```python
from build123d import *

# Parameters (mm, degrees)
BOSS_EXTRUDE1_DEPTH     = 240
CUT_EXTRUDE1_DEPTH      = 263.392835268
CUT_EXTRUDE2_DEPTH      = 263.392835268
CUT_EXTRUDE2_DEPTH_BACK = 263.392835268
SKETCH2_R               = 17.5
CHAMFER1_SIZE           = 4


with BuildPart() as part:
    # Sketch1 → Boss-Extrude1 (new, symmetric)
    with BuildSketch(Plane.XY):
        with BuildLine():
            Line((-63, -75), (63, -75))
            ThreePointArc((63, -75), (71.485281374, -71.485281374), (75, -63))
            Line((75, -63), (75, 63))
            ThreePointArc((75, 63), (71.485281374, 71.485281374), (63, 75))
            Line((63, 75), (-63, 75))
            ThreePointArc((-63, 75), (-71.485281374, 71.485281374), (-75, 63))
            Line((-75, 63), (-75, -63))
            ThreePointArc((-75, -63), (-71.485281374, -71.485281374), (-63, -75))
        make_face()
        with BuildLine():
            Line((-63, -69), (63, -69))
            ThreePointArc((63, -69), (67.242640687, -67.242640687), (69, -63))
            Line((69, -63), (69, 63))
            ThreePointArc((69, 63), (67.242640687, 67.242640687), (63, 69))
            Line((63, 69), (-63, 69))
            ThreePointArc((-63, 69), (-67.242640687, 67.242640687), (-69, 63))
            Line((-69, 63), (-69, -63))
            ThreePointArc((-69, -63), (-67.242640687, -67.242640687), (-63, -69))
        make_face(mode=Mode.SUBTRACT)
    extrude(amount=BOSS_EXTRUDE1_DEPTH, both=True)

    # 草图1 → Cut-Extrude1 (cut, through all)
    with BuildSketch(Plane(origin=(0, 0, 0), x_dir=(1, 0, 0), z_dir=(0, 1, 0))):
        with BuildLine():
            Line((40, -290), (-40, -290))
            Line((-40, -290), (-40, -200))
            ThreePointArc((-40, -200), (-37.071067812, -192.928932188), (-30, -190))
            Line((-30, -190), (30, -190))
            ThreePointArc((30, -190), (37.071067812, -192.928932188), (40, -200))
            Line((40, -200), (40, -290))
        make_face()
    extrude(amount=CUT_EXTRUDE1_DEPTH, mode=Mode.SUBTRACT)

    # Sketch2 → Cut-Extrude2 (cut, two sides: drawn at the far end of the back side and taken through both)
    with BuildSketch(Plane(origin=(0, 0, 0), x_dir=(0, 0, -1), z_dir=(1, 0, 0)).offset(-CUT_EXTRUDE2_DEPTH_BACK)):
        with Locations((-210, 0)):
            Circle(SKETCH2_R)
        with BuildLine():
            Line((200, 35), (285, 35))
            Line((285, 35), (285, -35))
            Line((285, -35), (200, -35))
            ThreePointArc((200, -35), (196.464466094, -33.535533906), (195, -30))
            Line((195, -30), (195, 30))
            ThreePointArc((195, 30), (196.464466094, 33.535533906), (200, 35))
        make_face()
    extrude(amount=CUT_EXTRUDE2_DEPTH + CUT_EXTRUDE2_DEPTH_BACK, mode=Mode.SUBTRACT)

    # Chamfer1
    chamfer1_edges = [part.edges().sort_by_distance(p)[0] for p in [
        (-67.242640687, 67.242640687, -240),
        (-69, 49, -240),
        (-67.242640687, -67.242640687, -240),
        (0, -69, -240),
        (67.242640687, -67.242640687, -240),
        (69, -49, -240),
        (67.242640687, 67.242640687, -240),
        (0, 69, -240),
        (69, 49, -240),
        (-69, -49, -240),
    ]]
    chamfer(chamfer1_edges, length=CHAMFER1_SIZE)


solid = part.part
```
Design review of the part built by this model. Coordinates are the model's own, in mm. A direction names the side the tool comes from. Round coordinates to 2 decimals unless told otherwise and drop trailing zeros. Order: outer loops, then holes, each group sorted by start corner. A loop starts at its lowest first (then second) coordinate and runs counter-clockwise, first axis right, second up. Notation, with made-up numbers: (13.25, 30.25) - (72.25, 30.25) arc R19 cw to (72.25, 55.25) - close; hole circle Ø5 at (-15, 88). An arc over 180 degrees is marked (long way). Return JSON: item names as keys, results as strings.
Q1. Consider section B-B on z = 210. Write out the cut boundary in (x, y), plus the area to 3 significant figures.
Computed values:
{"outline": "(-75, -63) arc R12 ccw to (-63, -75) - (63, -75) arc R12 ccw to (75, -63) - (75, -17.5) - (69, -17.5) - (69, -63) arc R6 cw to (63, -69) - (-63, -69) arc R6 cw to (-69, -63) - (-69, -17.5) - (-75, -17.5) - close; (-75, 17.5) - (-69, 17.5) - (-69, 63) arc R6 cw to (-63, 69) - (-40, 69) - (-40, 75) - (-63, 75) arc R12 ccw to (-75, 63) - close; (40, 69) - (63, 69) arc R6 cw to (69, 63) - (69, 17.5) - (75, 17.5) - (75, 63) arc R12 ccw to (63, 75) - (40, 75) - close", "area": "2,460 mm2"}
Q2. The part is to be moulded in two halves that separate along X. For faces 4 (the flat face through (0, 74, -240)), 5 (the flat face through (-1, -69, 5)), 6 (the conical face through (-68.3, 68.42, -237.58)), 7 (the flat face through (75, -1, 3)), say which applies: pulls with the +X half, pulls with the -X half, needs draft (parallel to the pull), parting line crosses it, or undercut.
Computed values:
{"face 4": "needs draft", "face 5": "undercut", "face 6": "undercut", "face 7": "pulls with the +X half"}
Q3. Consider section C-C on x = 2. Write out the cut boundary in (y, z), plus the area to 3 significant figures.
Computed values:
{"outline": "(-75, -240) - (-73, -240) - (-69, -236) - (-69, 240) - (-75, 240) - close; (69, -236) - (73, -240) - (75, -240) - (75, 190) - (69, 190) - close", "area": "5,440 mm2"}
Q4. Machinability: for faces 1 (the cylindrical face through (-37.15, 71.96, 193.01)), 2 (the flat face through (1, 69, 5)), 3 (the conical face through (68.42, 68.3, -237.58)), which of the approach directions +Z, -Z, +X, -X, +Y, -Y give a long, thin tool a straight path to every point of the face, cutting with its end or side? Answer none if there is none.
Computed values:
{"face 1": "+Z, +Y", "face 2": "+Z, -Z", "face 3": "-Z"}
Q5. Consider section D-D on y = -55.5. Write out the cut boundary in (x, z).
Computed values:
{"outline": "(-75, -240) - (-73, -240) - (-69, -236) - (-69, 240) - (-75, 240) - close; (69, -236) - (73, -240) - (75, -240) - (75, 240) - (69, 240) - close"}
Q6. Wall thickness on L1, parallel to Z at x = -73.2, y = 0; L2, parallel to Y at x = -38.5, z = -113: over which ranges is each line inside the solid? List them lowest first. Write a range as [from, to].
Computed values:
{"L1": "z = [-195, 192.5], [227.5, 240]", "L2": "y = [-75, -69], [69, 75]"}
Q7. Consider section A-A on y = 0. Write out the cut boundary in (x, z).
Computed values:
{"outline": "(-75, -195) - (-69, -195) - (-69, 192.5) - (-75, 192.5) - close; (-75, 227.5) - (-69, 227.5) - (-69, 240) - (-75, 240) - close; (69, -195) - (75, -195) - (75, 192.5) - (69, 192.5) - close; (69, 227.5) - (75, 227.5) - (75, 240) - (69, 240) - close"}
Q8. For pin 1 Ø1.8 at (x, z) = (-72.5, -225) entering from +Y; pin 2 Ø6.5 at (x, y) = (-72, 13.5) entering from -Z; pin 3 Ø5 at (x, z) = (-71.5, -218.5) entering from -Y; pin 4 Ø21 at (y, z) = (0, 210) entering from -X, all flat-tipped, find the tip position at first contact; note any pin that passes through.
Computed values:
{"pin 1": "stops at y = 71.37", "pin 2": "stops at z = -195", "pin 3": "stops at y = -73.39", "pin 4": "passes through"}
